from build123d import *

# Parameters (mm, degrees)
PLATE_PROFILE_SKETCH_R    = 4.065
BASE_PLATE_0_12IN_DEPTH   = 3.048
PLATE_EDGE_FILLET_R0_12_R = 3.048
HUB_SKETCH_0_5_R          = 6.35
HUB_0_5_X_1IN_DEPTH       = 25.4


with BuildPart() as part:
    # Plate Profile Sketch → Base Plate 0.12in (new body)
    with BuildSketch(Plane.XY):
        with BuildLine():
            Line((-19.05, 5.08), (-24.886815787, 5.08))
            ThreePointArc((-24.886815787, 5.08), (0, 25.4), (24.886815787, 5.08))
            Line((24.886815787, 5.08), (19.05, 5.08))
            ThreePointArc((19.05, 5.08), (13.97, 0), (19.05, -5.08))
            Line((19.05, -5.08), (24.886815787, -5.08))
            ThreePointArc((24.886815787, -5.08), (0, -25.4), (-24.886815787, -5.08))
            Line((-24.886815787, -5.08), (-19.05, -5.08))
            ThreePointArc((-19.05, -5.08), (-13.97, 0), (-19.05, 5.08))
        make_face()
        with Locations(Location((0, 19.05, 0), (0, 0, 180))):
            Circle(PLATE_PROFILE_SKETCH_R, mode=Mode.SUBTRACT)
        with Locations(Location((0, -19.05, 0), (0, 0, 180))):
            Circle(PLATE_PROFILE_SKETCH_R, mode=Mode.SUBTRACT)
    extrude(amount=BASE_PLATE_0_12IN_DEPTH)

    # Plate Edge Fillet R0.12
    plate_edge_fillet_r0_12_edges = [part.edges().sort_by_distance(p)[0] for p in [
        (-24.886815787, 5.08, 1.524),
        (24.886815787, 5.08, 1.524),
        (24.886815787, -5.08, 1.524),
        (-24.886815787, -5.08, 1.524),
    ]]
    fillet(plate_edge_fillet_r0_12_edges, radius=PLATE_EDGE_FILLET_R0_12_R)

    # Hub Sketch Ø0.5 → Hub Ø0.5 x 1in (add)
    with BuildSketch(Plane.XY.offset(3.048)):
        Circle(HUB_SKETCH_0_5_R)
    extrude(amount=HUB_0_5_X_1IN_DEPTH)

    # Sketch5 → Hub Tapped Hole #10-24 (revolve, cut)
    with BuildSketch(Plane(origin=(0, 0, 28.448), x_dir=(0, -1, 0), z_dir=(1, 0, 0))):
        Polygon((0, 0), (0, 26.472108517), (2.45, 25), (2.45, 23), (2.6, 23), (2.6, 0), align=None)
    revolve(axis=Axis((0, 0, 34.798), (0, 0, -1)), mode=Mode.SUBTRACT)


solid = part.part
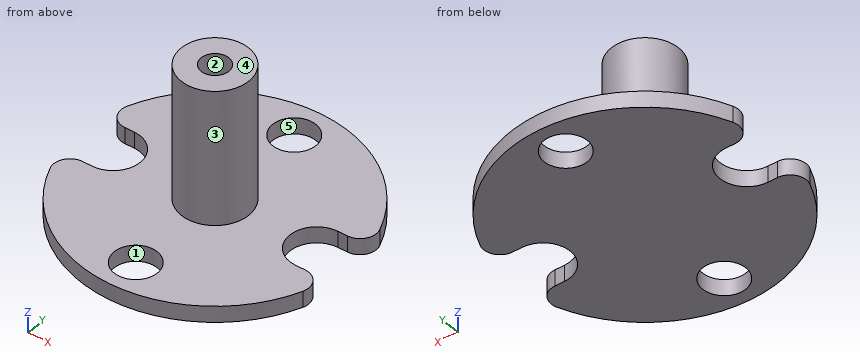
Check sheet for the modelled part. Datum: model origin and axes. Units: mm. Face numbers are marked on the shaded views. A direction names the side the tool comes from. Give positions to 0.01 mm unless a question says otherwise; leave off trailing zeros. Loops run counter-clockwise (first coordinate to the right, second up) from the corner with the lowest first, then second, coordinate; pieces in that order, holes last. Notation, with made-up numbers: M 12.25,76.5 L 38.25,76.5 A27 cw 38.25,113.5 Z; hole C 30.25,-1.5 d8. An arc over 180 degrees is marked long. Use a Markdown table: item, result. Add a question column.
Q1. Sectioned sample at C-C, the plane x = -5. Record the cut outline in (y, z), then the cut area to 3 significant figures.
Q2. Sectioned sample at B-B, the plane z = 14. Record the cut outline in (x, y).
Q3. Mould release check, pull along X, two halves, no side actions. Record for the marked faces 3, 4 and 5: pulls with the +X half, pulls with the -X half, needs draft (parallel to the pull), parting line crosses it, or undercut.
Q4. Go/stop test with flat-tipped pins: pin 1 (2 mm diameter, centred on x = 15, y = -3.5, fed in from +Z); pin 2 (0.5 mm diameter, centred on x = -20, z = 2, fed in from +Y); pin 3 (12 mm diameter, centred on y = -14, z = 7, fed in from +X). Record where each tip stops, or that it passes through.
Q5. Scan lines: line 1 along Z through (x, y) = (-21, -9.5); line 2 along X through (y, z) = (0.5, 5.75); line 3 along X through (y, z) = (19.05, 1) (3 decimals). Record each from-to range of solid material in increasing order. Write a range as [from, to].
Q6. Tool access check on the marked faces 1 and 2. Record the directions out of +Z, -Z, +X, -X, +Y, -Y that give a thin tool (end or side, any length) a straight path to the whole face; none if there is none.
Q7. Sectioned sample at A-A, the plane y = 19.05. Record the cut outline in (x, z) (3 decimals).
Verdict:
| question | item | result |
|---|---|---|
| 1 | outline | M -24.9,0 L 24.9,0 L 24.9,3.05 L 3.91,3.05 L 3.91,28.45 L -3.91,28.45 L -3.91,3.05 L -24.9,3.05 Z |
| 1 | area | 351 mm^2 |
| 2 | outline | C 0,0 d12.7; hole C 0,0 d5.2 |
| 3 | face 3 | parting line crosses it |
| 3 | face 4 | needs draft |
| 3 | face 5 | undercut |
| 4 | pin 1 | z = 3.05 |
| 4 | pin 2 | y = 15.97 |
| 4 | pin 3 | x = 23.56 |
| 5 | line 1 | [0, 3.05] |
| 5 | line 2 | [-6.33, -2.55], [2.55, 6.33] |
| 5 | line 3 | [-16.801, -4.065], [4.065, 16.801] |
| 6 | face 1 | +Z, -Z |
| 6 | face 2 | +Z |
| 7 | outline | M -16.801,0 L -4.065,0 L -4.065,3.048 L -16.801,3.048 Z; M 4.065,0 L 16.801,0 L 16.801,3.048 L 4.065,3.048 Z |
